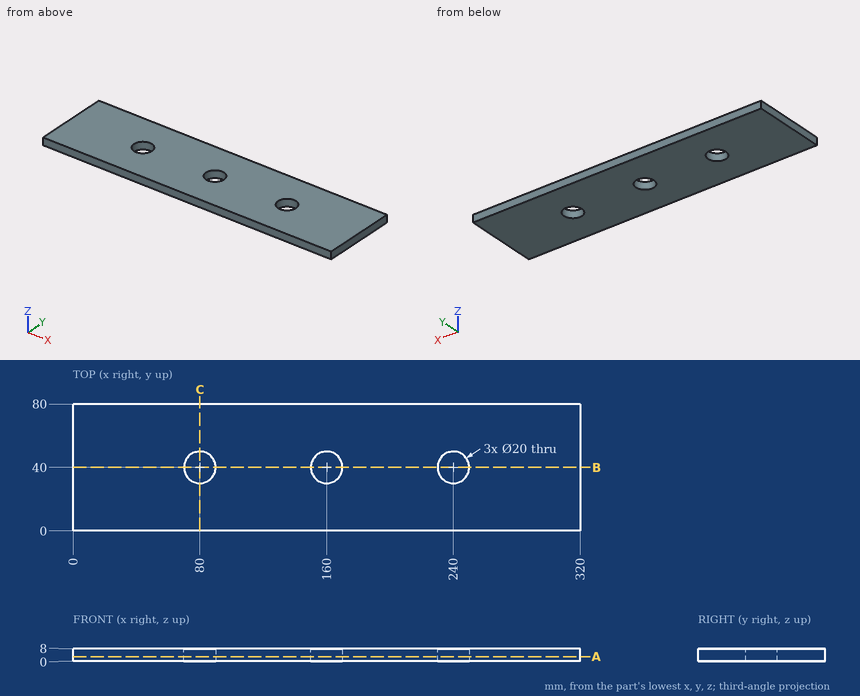
Design review of the part shown in the three views and the two pictorial views. Dimensions are in mm from the part's minimum x, y and z. Give positions to 0.01 mm unless a question says otherwise; leave off trailing zeros. Write each loop counter-clockwise with the first axis right and the second up, starting at its lowest first coordinate (ties: lowest second). Pieces come first, ordered by that corner, then holes. Notation, with made-up numbers: (-19.75, -14.5) -> (20.25, -14.5) arc R25 cw to (20.25, 14.5) -> close; hole circle Ø6 at (29.5, 25). An arc over 180 degrees is marked (long way). Answer in a Markdown table with one row per item.
1) Clearance check with a flat-ended pin moving along its axis: P1, Ø16, axis at x = 240, y = 40, coming from the -Z side. State where the tip first meets the part, or that it passes through.
Worked answers:
| item | result |
|---|---|
| P1 | through |
2) Add section B-B on y = 40. State the section outline as (x, z) points.
Worked answers:
| item | result |
|---|---|
| outline | (0, 0) -> (70, 0) -> (70, 8) -> (0, 8) -> close; (90, 0) -> (150, 0) -> (150, 8) -> (90, 8) -> close; (170, 0) -> (230, 0) -> (230, 8) -> (170, 8) -> close; (250, 0) -> (320, 0) -> (320, 8) -> (250, 8) -> close |
3) Add section C-C on x = 80. State the section outline as (y, z) points.
Worked answers:
| item | result |
|---|---|
| outline | (0, 0) -> (30, 0) -> (30, 8) -> (0, 8) -> close; (50, 0) -> (80, 0) -> (80, 8) -> (50, 8) -> close |
4) Add section A-A on z = 3. State the section outline as (x, y) points, plus the area to 3 significant figures.
Worked answers:
| item | result |
|---|---|
| outline | (0, 0) -> (320, 0) -> (320, 80) -> (0, 80) -> close; hole circle Ø20 at (80, 40); hole circle Ø20 at (160, 40); hole circle Ø20 at (240, 40) |
| area | 24,700 mm² |
5) For L1, parallel to X at y = 39, z = 3; L2, parallel to Y at x = 240, z = 6.25; L3, parallel to X at y = 48.5, z = 3.75, list the stretches that pass through material, from the lowest coordinate up. Write a range as [from, to].
Worked answers:
| item | result |
|---|---|
| L1 | [0, 70.05], [89.95, 150.05], [169.95, 230.05], [249.95, 320] |
| L2 | [0, 30], [50, 80] |
| L3 | [0, 74.73], [85.27, 154.73], [165.27, 234.73], [245.27, 320] |
